Could you check a few things on this model? Use its own coordinates, in mm. A direction names the side the tool comes from. Round coordinates to 2 decimals unless told otherwise and drop trailing zeros. Write each loop counter-clockwise with the first axis right and the second up, starting at its lowest first coordinate (ties: lowest second). Pieces come first, ordered by that corner, then holes. Notation, with made-up numbers: (19.25, 0) -> (35.25, 0) arc R27 cw to (35.25, 37) -> close; hole circle Ø7 at (47, 10). An arc over 180 degrees is marked (long way). Answer in a Markdown table with one row per item. Add a question column.
```python
from build123d import *

# Parameters (mm, degrees)
BASE_PLATE_DEPTH              = 7
BASE_RELIEF_CUT_DEPTH         = 16
BASE_RELIEF_CUT_DEPTH_BACK    = 18
BASE_RELIEF_CUT_SKETCH_R      = 3.5
BASE_TRIM_CUT_DEPTH           = 27
BASE_TRIM_CUT_DEPTH_BACK      = 35
BASE_TRIM_CUT_SKETCH_R        = 3.5
UPRIGHT_BLOCK_SKETCH_13X13_W  = 25.796955258
UPRIGHT_BLOCK_SKETCH_13X13_H  = 16
UPRIGHT_BLOCK_DEPTH           = 25
UPRIGHT_SLOT_DEPTH            = 38
UPRIGHT_SLOT_DEPTH_BACK       = 84
UPRIGHT_CROSS_HOLE_DEPTH      = 10
UPRIGHT_CROSS_HOLE_DEPTH_BACK = 13
UPRIGHT_CROSS_HOLE_SKETCH_R   = 3.5
THROUGH_HOLE_SKETCH_R         = 3.5
THROUGH_HOLE_DEPTH            = 14
BASE_CLEARANCE_CUT_DEPTH      = 17
BASE_CLEARANCE_CUT_DEPTH_BACK = 58
BASE_CLEARANCE_CUT_SKETCH_W   = 13
BASE_CLEARANCE_CUT_SKETCH_H   = 9


with BuildPart() as part:
    # Base Plate Sketch → Base Plate (new body)
    with BuildSketch(Plane(origin=(0, 0, 0), x_dir=(1, 0, 0), z_dir=(0, 1, 0))):
        Polygon((-51.796955258, -2.197106083), (-51.796955258, -12.197106083), (-45.898477629, -18.197106083), (-5.898477629, -18.197106083), (0, -12.197106083), (0, -2.197106083), align=None)
    extrude(amount=BASE_PLATE_DEPTH)

    # Base Relief Cut Sketch → Base Relief Cut (cut, two sides: drawn at the far end of the back side and taken through both)
    with BuildSketch(Plane(origin=(0, 7, 0), x_dir=(1, 0, 0), z_dir=(0, 1, 0)).offset(-BASE_RELIEF_CUT_DEPTH_BACK)):
        with Locations(Location((-45.296955258, -9.519706742, 0), (0, 0, 270))):
            Circle(BASE_RELIEF_CUT_SKETCH_R)
    extrude(amount=BASE_RELIEF_CUT_DEPTH + BASE_RELIEF_CUT_DEPTH_BACK, mode=Mode.SUBTRACT)

    # Base Trim Cut Sketch → Base Trim Cut (cut, two sides: drawn at the far end of the back side and taken through both)
    with BuildSketch(Plane(origin=(0, 7, 0), x_dir=(1, 0, 0), z_dir=(0, 1, 0)).offset(-BASE_TRIM_CUT_DEPTH_BACK)):
        with Locations(Location((-6.250512003, -9.218640368, 0), (0, 0, 270))):
            Circle(BASE_TRIM_CUT_SKETCH_R)
    extrude(amount=BASE_TRIM_CUT_DEPTH + BASE_TRIM_CUT_DEPTH_BACK, mode=Mode.SUBTRACT)

    # Upright Block Sketch 13x13 → Upright Block (add)
    with BuildSketch(Plane(origin=(0, 7, 0), x_dir=(1, 0, 0), z_dir=(0, 1, 0))):
        with Locations((-25.898477629, -10.197106083)):
            Rectangle(UPRIGHT_BLOCK_SKETCH_13X13_W, UPRIGHT_BLOCK_SKETCH_13X13_H)
    extrude(amount=UPRIGHT_BLOCK_DEPTH)

    # Upright Slot Sketch → Upright Slot (cut, two sides: drawn at the far end of the back side and taken through both)
    with BuildSketch(Plane.XY.offset(18.197106083).offset(-UPRIGHT_SLOT_DEPTH_BACK)):
        Polygon((-28.796955258, 32), (-28.796955258, 22.247127252), (-28.796955258, 14), (-23, 14), (-23, 32), align=None)
    extrude(amount=UPRIGHT_SLOT_DEPTH + UPRIGHT_SLOT_DEPTH_BACK, mode=Mode.SUBTRACT)

    # Upright Cross Hole Sketch → Upright Cross Hole (cut, two sides: drawn at the far end of the back side and taken through both)
    with BuildSketch(Plane(origin=(-13, 0, 0), x_dir=(0, 0, -1), z_dir=(1, 0, 0)).offset(-UPRIGHT_CROSS_HOLE_DEPTH_BACK)):
        with Locations(Location((-10.197106083, 22, 0), (0, 0, 270))):
            Circle(UPRIGHT_CROSS_HOLE_SKETCH_R)
    extrude(amount=UPRIGHT_CROSS_HOLE_DEPTH + UPRIGHT_CROSS_HOLE_DEPTH_BACK, mode=Mode.SUBTRACT)

    # Through Hole Sketch → Through Hole (cut)
    with BuildSketch(Plane(origin=(-28.796955258, 0, 0), x_dir=(0, 0, -1), z_dir=(1, 0, 0))):
        with Locations(Location((-10.197106083, 22, 0), (0, 0, 270))):
            Circle(THROUGH_HOLE_SKETCH_R)
    extrude(amount=-THROUGH_HOLE_DEPTH, mode=Mode.SUBTRACT)

    # Base Clearance Cut Sketch → Base Clearance Cut (cut, two sides: drawn at the far end of the back side and taken through both)
    with BuildSketch(Plane.XY.offset(18.197106083).offset(-BASE_CLEARANCE_CUT_DEPTH_BACK)):
        with Locations((-25.898477629, 4.5)):
            Rectangle(BASE_CLEARANCE_CUT_SKETCH_W, BASE_CLEARANCE_CUT_SKETCH_H)
    extrude(amount=BASE_CLEARANCE_CUT_DEPTH + BASE_CLEARANCE_CUT_DEPTH_BACK, mode=Mode.SUBTRACT)


solid = part.part
```
(1) Suppose I cut it at C-C, the plane y = 6. Please give me the cut outline in (x, z).
(2) Suppose I cut it at A-A, the plane y = 22. Please give me the cut outline in (x, z).
(3) If we mould it in two halves opening along X, with no side actions, what happens to faces 4 (the face through (-26, 9, 10)), 5 (the face through (-33.73, 18.66, 9.15)), 6 (the face through (0, 3, 7))? For each: pulls with the +X half, pulls with the -X half, needs draft (parallel to the pull), parting line crosses it, or undercut.
(4) For P1, Ø2, axis at y = 12, z = 7, coming from the -X side; P2, Ø6.5, axis at x = -44.5, z = 11.5, coming from the +Y side; P3, Ø6.5, axis at x = -24.5, z = 7, coming from the -Y side, each with a flat end and sliding along its axis, tell me the tip position at first contact or that it passes through.
(5) Suppose I cut it at D-D, the plane z = 9.5. State how many separate pieces and enclosed holes the cut face has, then the cut area to 3 significant figures.
(6) I need wall thicknesses on L1, parallel to X at y = 15, z = 4; L2, parallel to Z at x = -16, y = 22; L3, parallel to X at y = 4.5, z = 9. Which ranges of each line are inside material? Lowest first, please.
(7) On a 3-axis mill with a long thin cutter (end or side, diameter ignored), from which of +Z, -Z, +X, -X, +Y, -Y can I reach the whole of each face in a straight line? I mean faces 1 (the face through (-23, 23, 14)), 2 (the face through (-19.398, 4, 10)), 3 (the face through (-9, 7, 12)). Say none if no direction works.
(8) Suppose I cut it at B-B, the plane z = 4.75. Please give me the cut outline in (x, y), then the cut area to 3 significant figures.
Response:
| question | item | result |
|---|---|---|
| 1 | outline | (-51.8, 2.2) -> (-32.4, 2.2) -> (-32.4, 18.2) -> (-45.9, 18.2) -> (-51.8, 12.2) -> close; (-19.4, 2.2) -> (0, 2.2) -> (0, 12.2) -> (-5.9, 18.2) -> (-19.4, 18.2) -> close; hole circle Ø7 at (-45.3, 9.52); hole circle Ø7 at (-6.25, 9.22) |
| 2 | outline | (-38.8, 2.2) -> (-28.8, 2.2) -> (-28.8, 6.7) -> (-38.8, 6.7) -> close; (-38.8, 13.7) -> (-28.8, 13.7) -> (-28.8, 18.2) -> (-38.8, 18.2) -> close; (-23, 2.2) -> (-13, 2.2) -> (-13, 6.7) -> (-23, 6.7) -> close; (-23, 13.7) -> (-13, 13.7) -> (-13, 18.2) -> (-23, 18.2) -> close |
| 3 | face 4 | undercut |
| 3 | face 5 | needs draft |
| 3 | face 6 | pulls with the +X half |
| 4 | P1 | x = -38.8 |
| 4 | P2 | y = 7 |
| 4 | P3 | y = 9 |
| 5 | separate pieces | 5 |
| 5 | enclosed holes | 0 |
| 5 | area | 551 mm² |
| 6 | L1 | -38.8 to -28.8, -23 to -13 |
| 6 | L2 | 2.2 to 6.7, 13.7 to 18.2 |
| 6 | L3 | -51.8 to -48.76, -41.84 to -32.4, -19.4 to -9.74, -2.76 to 0 |
| 7 | face 1 | +Z, -Z, +Y |
| 7 | face 2 | +Z, -Z, -Y |
| 7 | face 3 | +Z, -Z, +X, +Y |
| 8 | outline | (-51.8, 0) -> (-32.4, 0) -> (-32.4, 9) -> (-19.4, 9) -> (-19.4, 0) -> (0, 0) -> (0, 7) -> (-13, 7) -> (-13, 32) -> (-23, 32) -> (-23, 14) -> (-28.8, 14) -> (-28.8, 32) -> (-38.8, 32) -> (-38.8, 7) -> (-51.8, 7) -> close |
| 8 | area | 786 mm² |
